Geometry: final body of the model. Coordinates: model frame, mm. Round coordinates to 2 decimals unless told otherwise and drop trailing zeros. Write each loop counter-clockwise with the first axis right and the second up, starting at its lowest first coordinate (ties: lowest second). Pieces come first, ordered by that corner, then holes. Notation, with made-up numbers: (-18, 11) - (-10, 11) arc R17 ccw to (-10, 32) - close; hole circle Ø4 at (-31, 77). An arc over 180 degrees is marked (long way). Write each question's results on one line, items separated by ' | '.
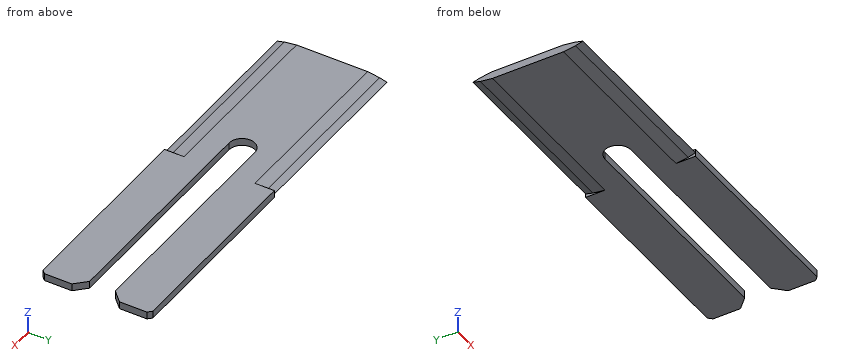
from build123d import *

# Parameters (mm, degrees)
SKETCH_2_W               = 105
SKETCH_2_H               = 30
EXTRUDE_1_DEPTH          = 2
CUT_EXTRUDE_1_DEPTH      = 55.637441375
CUT_EXTRUDE_1_DEPTH_BACK = 55.637441375
SKETCH_5_OUTSIDE_W       = 25.844
SKETCH_5_OUTSIDE_H       = 53.844
CUT_EXTRUDE_7_DEPTH      = 50
CHAMFER_1_SIZE           = 1
CHAMFER_2_SIZE           = 3


with BuildPart() as part:
    # 草图2 → 凸台-拉伸1 (new body)
    with BuildSketch(Plane.XY):
        Rectangle(SKETCH_2_W, SKETCH_2_H)
    extrude(amount=EXTRUDE_1_DEPTH)

    # 草图3 → 切除-拉伸1 (cut, two sides: drawn at the far end of the back side and taken through both)
    with BuildSketch(Plane.XY.offset(2).offset(-CUT_EXTRUDE_1_DEPTH_BACK)):
        with BuildLine():
            Line((52.5, 3.5), (-12.5, 3.5))
            ThreePointArc((-12.5, 3.5), (-16, 0), (-12.5, -3.5))
            Line((-12.5, -3.5), (52.5, -3.5))
            Line((52.5, -3.5), (52.5, 3.5))
        make_face()
    extrude(amount=CUT_EXTRUDE_1_DEPTH + CUT_EXTRUDE_1_DEPTH_BACK, mode=Mode.SUBTRACT)

    # 草图5 outside → 切除-拉伸7 (cut)
    with BuildSketch(Plane.ZY.offset(52.5)):
        with Locations((1, 0)):
            Rectangle(SKETCH_5_OUTSIDE_W, SKETCH_5_OUTSIDE_H)
        Polygon((1, 15), (0.464101615, 13), (0, 9.69774542), (0, -9.69774542), (0.464101615, -13), (1, -15), (1.535898385, -13), (2, -9.69774542), (2, 9.69774542), (1.535898385, 13), align=None, mode=Mode.SUBTRACT)
    extrude(amount=-CUT_EXTRUDE_7_DEPTH, mode=Mode.SUBTRACT)

    # 倒角1
    chamfer_1_edges = [part.edges().sort_by_distance(p)[0] for p in [
        (52.5, -15, 1),
        (52.5, 15, 1),
    ]]
    chamfer(chamfer_1_edges, length=CHAMFER_1_SIZE)

    # 倒角2
    chamfer_2_edges = [part.edges().sort_by_distance(p)[0] for p in [
        (52.5, -3.5, 1),
        (52.5, 3.5, 1),
    ]]
    chamfer(chamfer_2_edges, length=CHAMFER_2_SIZE)


solid = part.part
Q1. Section query C-C, the plane y = -11.75. Return loops of the section in (x, z), plus the area to 3 significant figures.
Answer block:
outline: (-52.5, 0.29) - (-2.5, 0.29) - (-2.5, 0) - (52.5, 0) - (52.5, 2) - (-2.5, 2) - (-2.5, 1.71) - (-52.5, 1.71) - close | area: 181 mm2
Q2. Section query A-A, the plane x = 19.5. Return loops of the section in (y, z).
Answer block:
outline: (-15, 0) - (-3.5, 0) - (-3.5, 2) - (-15, 2) - close; (3.5, 0) - (15, 0) - (15, 2) - (3.5, 2) - close
Q3. Section query D-D, the plane y = 0. Return loops of the section in (x, z), plus the area to 3 significant figures.
Answer block:
outline: (-52.5, 0) - (-16, 0) - (-16, 2) - (-52.5, 2) - close | area: 73.0 mm2
Q4. Section query B-B, the plane x = -36. Return loops of the section in (y, z), plus the area to 3 significant figures.
Answer block:
outline: (-15, 1) - (-13, 0.46) - (-9.7, 0) - (9.7, 0) - (13, 0.46) - (15, 1) - (13, 1.54) - (9.7, 2) - (-9.7, 2) - (-13, 1.54) - close | area: 51.1 mm2
Q5. Ray query, line 1 along Y through (x, z) = (28.5, 0.35); line 2 along X through (y, z) = (12, 1.75); line 3 along Z through (x, y) = (-17, 9.75). Return the intervals inside material, ascending.
Answer block:
line 1: -15 to -3.5, 3.5 to 15 | line 2: -2.5 to 52.5 | line 3: 0.01 to 1.99
